For this review, take the finished solid that the model builds, in its own axes (mm). Face numbers are marked on the shaded views. A direction names the side the tool comes from. Round coordinates to 2 decimals unless told otherwise and drop trailing zeros. Order: outer loops, then holes, each group sorted by start corner. A loop starts at its lowest first (then second) coordinate and runs counter-clockwise, first axis right, second up.
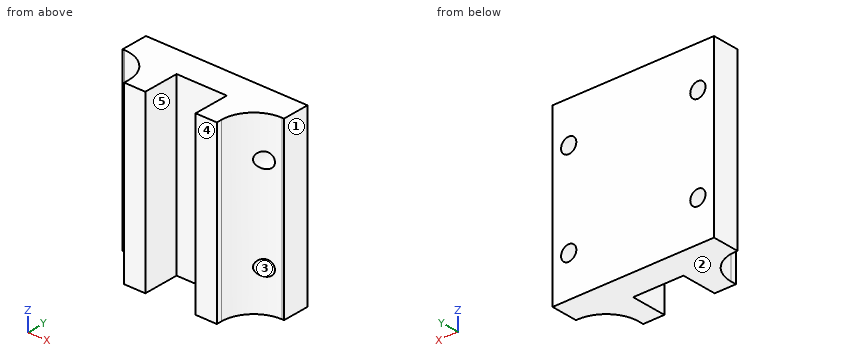
from build123d import *

# Parameters (mm, degrees)
BOSS_EXTRUDE1_DEPTH    = 48.7
M10_TAPPED_HOLE1_D     = 8.5
M10_TAPPED_HOLE1_DEPTH = 24.5
M10_TAPPED_HOLE1_TIP   = 2.553657631


with BuildPart() as part:
    # Sketch1 → Boss-Extrude1 (new, symmetric)
    with BuildSketch(Plane.XY):
        with BuildLine():
            Line((-25.830388506, -36), (-25.830388506, -33))
            ThreePointArc((-25.830388506, -33), (-31.102466444, -20.272077939), (-43.830388506, -15))
            Line((-43.830388506, -15), (-45, -15))
            Line((-45, -15), (-45, 0))
            Line((-45, 0), (45, 0))
            Line((45, 0), (45, -15))
            Line((45, -15), (43.830388506, -15))
            ThreePointArc((43.830388506, -15), (31.102466444, -20.272077939), (25.830388506, -33))
            Line((25.830388506, -33), (25.830388506, -36))
            Line((25.830388506, -36), (14, -36))
            Line((14, -36), (14, -16))
            Line((14, -16), (-14, -16))
            Line((-14, -16), (-14, -36))
            Line((-14, -36), (-25.830388506, -36))
        make_face()
    extrude(amount=BOSS_EXTRUDE1_DEPTH, both=True)

    # M10 Tapped Hole1
    with Locations(Plane(origin=(0, 0, 0), x_dir=(-1, 0, 0), z_dir=(0, 1, 0))):
        with Locations((-36, 26), (36, 26), (-36, -26), (36, -26)):
            Hole(M10_TAPPED_HOLE1_D / 2, depth=M10_TAPPED_HOLE1_DEPTH)
            with Locations((0, 0, -(M10_TAPPED_HOLE1_DEPTH + M10_TAPPED_HOLE1_TIP / 2))):  # 118° drill point
                Cone(0, M10_TAPPED_HOLE1_D / 2, M10_TAPPED_HOLE1_TIP, mode=Mode.SUBTRACT)


solid = part.part
(1) Add section D-D on y = -12. Give the boundary of the cut face in (x, z), plus the area to 3 significant figures.
(2) Tool access review of the marked faces 4 and 5: name each direction out of +Z, -Z, +X, -X, +Y, -Y from which nothing blocks a thin tool from reaching the whole face with its end or side.
(3) Clearance check with flat-ended pins moving along their axes: P1, Ø16, axis at y = -26, z = -14.5, coming from the -X side; P2, Ø2.5, axis at y = -34, z = -5.5, coming from the +X side; P3, Ø1.5, axis at y = -25.5, z = 18.5, coming from the +X side. State where each tip first meets the part, or that it passes through.
(4) Add section C-C on x = -34.5. Give the boundary of the cut face in (y, z).
(5) Wall thickness on L1, parallel to X at y = -5.25, z = 26; L2, parallel to Z at x = -36, y = -6; L3, parallel to Y at x = -9.5, z = -16.5: over which ranges is each line inside the solid? List them lowest first.
(6) Add section B-B on y = -31.5. Give the boundary of the cut face in (x, z).
(7) Draft analysis for pull direction Z (two halves, no side actions). For the marked faces 1, 2 and 3, state which applies: pulls with the +Z half, pulls with the -Z half, needs draft (parallel to the pull), parting line crosses it, or undercut.
(8) Add section A-A on z = -17. Give the boundary of the cut face in (x, y).
Here are the results:
1. outline: (-45, -48.7) - (45, -48.7) - (45, 48.7) - (-45, 48.7) - close; hole circle Ø8.5 at (-36, -26); hole circle Ø8.5 at (-36, 26); hole circle Ø8.5 at (36, -26); hole circle Ø8.5 at (36, 26)
1. area: 8,540 mm2
2. face 4: +Z, -Z, +X, -X, -Y
2. face 5: +Z, -Z, -Y
3. P1: stops at x = -33.88
3. P2: stops at x = 25.83
3. P3: stops at x = 27.83
4. outline: (-17.61, -48.7) - (0, -48.7) - (0, -29.98) - (-17.61, -29.98) - close; (-17.61, -22.02) - (0, -22.02) - (0, 22.02) - (-17.61, 22.02) - close; (-17.61, 29.98) - (0, 29.98) - (0, 48.7) - (-17.61, 48.7) - close
5. L1: x = -45 to -40.25, -31.75 to 31.75, 40.25 to 45
5. L2: z = -48.7 to -30.25, -21.75 to 21.75, 30.25 to 48.7
5. L3: y = -16 to 0
6. outline: (-25.89, -48.7) - (-14, -48.7) - (-14, 48.7) - (-25.89, 48.7) - close; (14, -48.7) - (25.89, -48.7) - (25.89, 48.7) - (14, 48.7) - close
7. face 1: needs draft
7. face 2: pulls with the -Z half
7. face 3: undercut
8. outline: (-45, -15) - (-43.83, -15) arc R18 cw to (-25.83, -33) - (-25.83, -36) - (-14, -36) - (-14, -16) - (14, -16) - (14, -36) - (25.83, -36) - (25.83, -33) arc R18 cw to (43.83, -15) - (45, -15) - (45, 0) - (-45, 0) - close
